Can you work these out from the drawing? Everything is in mm from the part's minimum corner. Coordinates: 2 decimals unless noted, no trailing zeros. Order: outer loops, then holes, each group sorted by start corner. A loop starts at its lowest first (then second) coordinate and runs counter-clockwise, first axis right, second up. Notation, with made-up numbers: (35, 46.25) -> (91, 46.25) arc R27 ccw to (91, 82.25) -> close; hole circle Ø2 at (66, 42). An arc over 180 degrees is marked (long way). Return JSON: item names as keys, results as strings. Group by question number.
1) For pin 1 (11.5 mm diameter, centred on y = 900, z = 319.5, fed in from +X); pin 2 (12 mm diameter, centred on y = 859.5, z = 588, fed in from +X); pin 3 (1 mm diameter, centred on y = 849.5, z = 509.5, fed in from +X), each with a flat end and sliding along its axis, tell me the tip position at first contact or that it passes through.
2) Thinking about a two-plate mould opening in Y: for the marked faces 1 and 2, which applies, +Y half, -Y half, draft (parallel to the pull), parting line (faces both ways), or undercut?
3) If we section it at D-D, the plane x = 761.5: Please give me the cut outline in (y, z).
4) If we section it at A-A, the plane z = 395.5: Please give me the cut outline in (x, y), then the cut area to 3 significant figures.
5) If I drill on probe 1 along Y at (x, z) = (485, 433); probe 2 along Y at (x, z) = (722, 272.5); probe 3 along X at (y, z) = (282.5, 511.5), over which ranges is the centre line in solid material (lowest first)? Write a range as from..to.
6) If we section it at B-B, the plane x = 485: Please give me the cut outline in (y, z), then the cut area to 3 significant figures.
7) If we section it at C-C, the plane y = 485: Please give me the cut outline in (x, z).
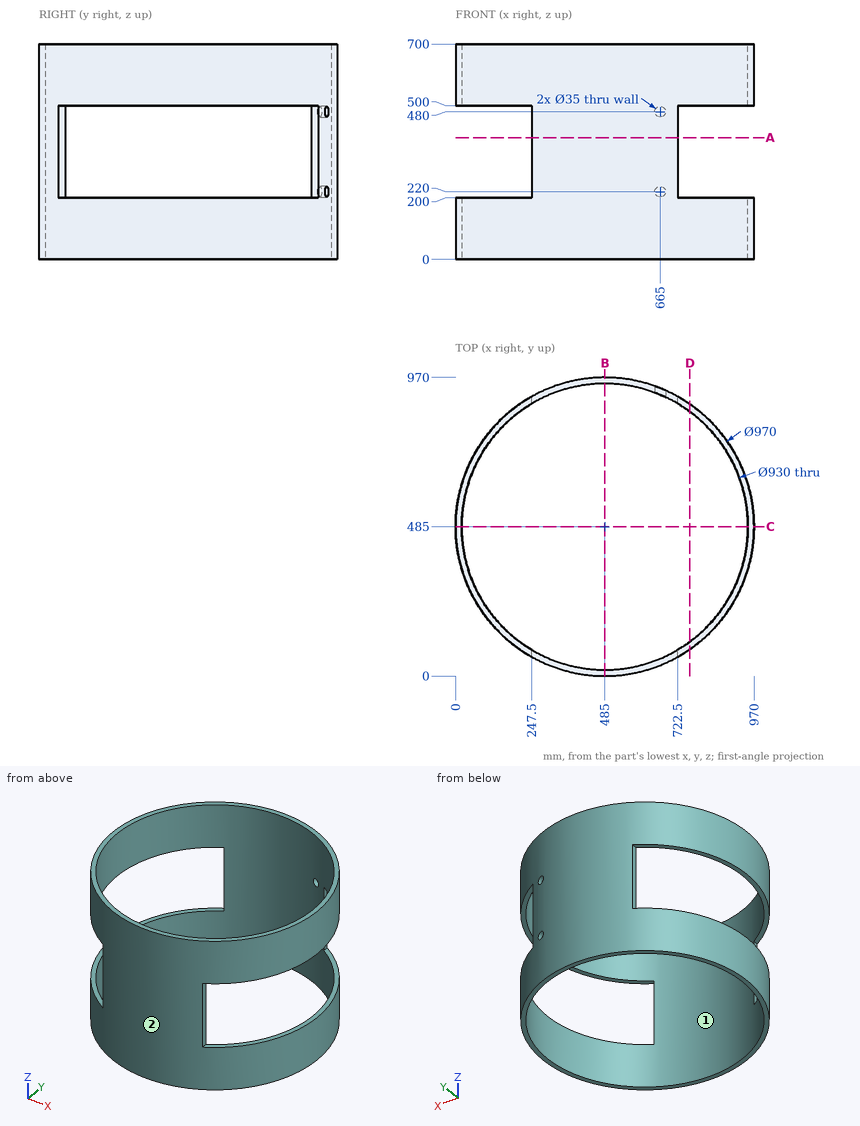
Result sheet:
{
 "1": {"pin 1": "stops at x = 722.5", "pin 2": "stops at x = 800.33", "pin 3": "stops at x = 805.51"},
 "2": {"face 1": "undercut", "face 2": "parting line"},
 "3": {"outline": "(86.54, 0) -> (111.14, 0) -> (111.14, 200) -> (86.54, 200) -> close; (86.54, 500) -> (111.14, 500) -> (111.14, 700) -> (86.54, 700) -> close; (858.86, 0) -> (883.46, 0) -> (883.46, 200) -> (858.86, 200) -> close; (858.86, 500) -> (883.46, 500) -> (883.46, 700) -> (858.86, 700) -> close"},
 "4": {"outline": "(247.5, 62.13) arc R485 ccw to (722.5, 62.13) -> (722.5, 85.23) arc R465 cw to (247.5, 85.23) -> close; (247.5, 884.77) arc R465 cw to (722.5, 884.77) -> (722.5, 907.87) arc R485 ccw to (247.5, 907.87) -> close", "area": "19,900 mm2"},
 "5": {"probe 1": "y = 0..20, 950..970", "probe 2": "y = 61.85..84.93, 885.07..908.15", "probe 3": "x = 44.3..66.41, 903.59..925.7"},
 "6": {"outline": "(0, 0) -> (20, 0) -> (20, 700) -> (0, 700) -> close; (950, 0) -> (970, 0) -> (970, 700) -> (950, 700) -> close", "area": "28,000 mm2"},
 "7": {"outline": "(0, 0) -> (20, 0) -> (20, 200) -> (0, 200) -> close; (0, 500) -> (20, 500) -> (20, 700) -> (0, 700) -> close; (950, 0) -> (970, 0) -> (970, 200) -> (950, 200) -> close; (950, 500) -> (970, 500) -> (970, 700) -> (950, 700) -> close"}
}
